from build123d import *

# Parameters (mm, degrees)
SKETCH_1_R      = 32.500096928
EXTRUDE_1_DEPTH = 40
SKETCH_2_R      = 47.5
SKETCH_2_R_2    = 32.5
EXTRUDE_2_DEPTH = 5


with BuildPart() as part:
    # 草图1 → 凸台-拉伸1 (new body)
    with BuildSketch(Plane(origin=(0, 0, 0), x_dir=(1, 0, 0), z_dir=(0, 1, 0))):
        with Locations(Location((0, 0, 0), (0, 0, 270))):
            Circle(SKETCH_1_R)
        with BuildLine():
            Line((0, 20.591616466), (5, 20.591616466))
            Line((5, 20.591616466), (5, 17.291616466))
            ThreePointArc((5, 17.291616466), (18, 0), (5, -17.291616466))
            Line((5, -17.291616466), (5, -20.591616466))
            Line((5, -20.591616466), (0, -20.591616466))
            Line((0, -20.591616466), (-5, -20.591616466))
            Line((-5, -20.591616466), (-5, -17.291616466))
            ThreePointArc((-5, -17.291616466), (-18, 0), (-5, 17.291616466))
            Line((-5, 17.291616466), (-5, 20.591616466))
            Line((-5, 20.591616466), (0, 20.591616466))
        make_face(mode=Mode.SUBTRACT)
    extrude(amount=EXTRUDE_1_DEPTH)

    # 草图2 → 凸台-拉伸2 (add)
    with BuildSketch(Plane.XZ):
        with Locations(Location((0, 0, 0), (0, 0, 270))):
            Circle(SKETCH_2_R)
        Circle(SKETCH_2_R_2, mode=Mode.SUBTRACT)
    extrude(amount=-EXTRUDE_2_DEPTH)


solid = part.part
Input: part model. Units: mm. Frame: model coordinates. A direction names the side the tool comes from. Round coordinates to 2 decimals unless told otherwise and drop trailing zeros. Write each loop counter-clockwise with the first axis right and the second up, starting at its lowest first coordinate (ties: lowest second). Pieces come first, ordered by that corner, then holes.
1) Contact query for flat-ended pins moving along their axis: P1, Ø1.5, axis at x = 31, z = -14, coming from the +Y side; P2, Ø1.7, axis at y = 23.5, z = -19, coming from the +X side; P3, Ø3, axis at x = 1.5, y = 21.5, coming from the -Z side. Output: stop coordinate, or through.
2) Cut plane C-C (z = 0). Return the cut outline in (x, y), then the cut area to 3 significant figures.
3) Draft query along Z for faces 1 (the cylindrical face through (-19.78, 22.26, -25.79)), 2 (the flat face through (5, 20, 19)), 3 (the flat face through (-14, 40, 14)), 4 (the flat face through (0, 20, 20.592)). Return one class per face: pulls with the +Z half, pulls with the -Z half, needs draft (parallel to the pull), parting line crosses it, or undercut.
4) Reachability of faces 5 (the flat face through (11, 5, -31)), 6 (the cylindrical face through (18, 20, 0)), 7 (the flat face through (-20, 0, 1)) from +Z, -Z, +X, -X, +Y, -Y: full face, straight path, thin tool, end or side. Return the list, or none.
5) Cut plane D-D (y = 3). Return the cut outline in (x, z), then the cut area to 3 significant figures.
6) Ray query, L1, parallel to X at y = 15.5, z = -11; L2, parallel to Y at x = 5.5, z = 38; L3, parallel to X at y = 14, z = 16.5. Return the intervals inside material, ascending.
7) Cut plane B-B (x = 0). Return the cut outline in (y, z).
8) Cut plane A-A (y = 18). Return the cut outline in (x, z), then the cut area to 3 significant figures.
Geometry says:
1. P1: stops at y = 5
1. P2: stops at x = 26.96
1. P3: stops at z = -32.5
2. outline: (-47.5, 0) - (-18, 0) - (-18, 40) - (-32.5, 40) - (-32.5, 5) - (-47.5, 5) - close; (18, 0) - (47.5, 0) - (47.5, 5) - (32.5, 5) - (32.5, 40) - (18, 40) - close
2. area: 1,310 mm2
3. face 1: parting line crosses it
3. face 2: undercut
3. face 3: needs draft
3. face 4: undercut
4. face 5: +Y
4. face 6: +Y, -Y
4. face 7: +Z, -Z, +X, -X, -Y
5. outline: circle Ø95 at (0, 0); hole (-5, -20.59) - (5, -20.59) - (5, -17.29) arc R18 ccw to (5, 17.29) - (5, 20.59) - (-5, 20.59) - (-5, 17.29) arc R18 ccw to (-5, -17.29) - close
5. area: 6,010 mm2
6. L1: x = -30.58 to -14.25, 14.25 to 30.58
6. L2: y = 0 to 5
6. L3: x = -28 to -7.19, 7.19 to 28
7. outline: (0, -47.5) - (5, -47.5) - (5, -32.5) - (40, -32.5) - (40, -20.59) - (0, -20.59) - close; (0, 20.59) - (40, 20.59) - (40, 32.5) - (5, 32.5) - (5, 47.5) - (0, 47.5) - close
8. outline: circle Ø65 at (0, 0); hole (-5, -20.59) - (5, -20.59) - (5, -17.29) arc R18 ccw to (5, 17.29) - (5, 20.59) - (-5, 20.59) - (-5, 17.29) arc R18 ccw to (-5, -17.29) - close
8. area: 2,240 mm2
